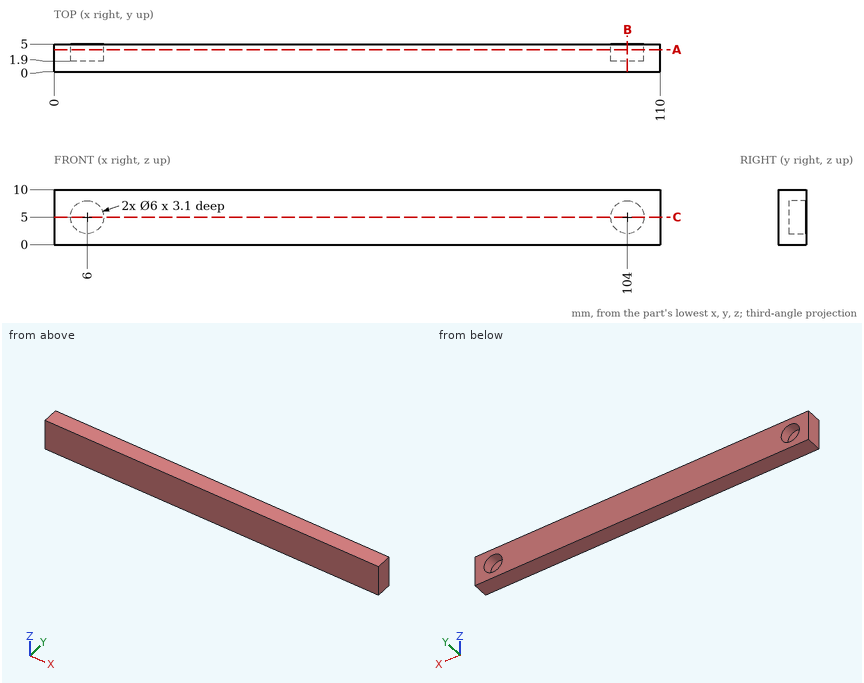
Could you check a few things on this drawing? It's one solid part, dimensions in mm from its lowest x, y, z. Round coordinates to 2 decimals unless told otherwise and drop trailing zeros. Write each loop counter-clockwise with the first axis right and the second up, starting at its lowest first coordinate (ties: lowest second). Pieces come first, ordered by that corner, then holes.
Q1. If we section it at B-B on x = 104: Write out the boundary of the cut face in (y, z).
Q2. If we section it at C-C on z = 5: Write out the boundary of the cut face in (x, y), plus the area to 3 significant figures.
Q3. Please list where these lines run through material, in increasing order: probe 1 along X at (y, z) = (2.7, 5); probe 2 along X at (y, z) = (4.4, 2.5); probe 3 along Z at (x, y) = (6.5, 3.75).
Q4. If we section it at A-A on y = 4: Write out the boundary of the cut face in (x, z).
Q5. Will these pins go through, and if not, where does the flat tip stop? P1, Ø1, axis at y = 4, z = 2.5, coming from the -X side; P2, Ø3, axis at x = 7, z = 6, coming from the +Y side.
Answer below:
1. outline: (0, 0) - (5, 0) - (5, 2) - (1.9, 2) - (1.9, 8) - (5, 8) - (5, 10) - (0, 10) - close
2. outline: (0, 0) - (110, 0) - (110, 5) - (107, 5) - (107, 1.9) - (101, 1.9) - (101, 5) - (9, 5) - (9, 1.9) - (3, 1.9) - (3, 5) - (0, 5) - close
2. area: 513 mm2
3. probe 1: x = 0 to 3, 9 to 101, 107 to 110
3. probe 2: x = 0 to 4.34, 7.66 to 102.34, 105.66 to 110
3. probe 3: z = 0 to 2.04, 7.96 to 10
4. outline: (0, 0) - (110, 0) - (110, 10) - (0, 10) - close; hole circle Ø6 at (6, 5); hole circle Ø6 at (104, 5)
5. P1: stops at x = 0
5. P2: stops at y = 1.9
